```python
from build123d import *

# Parameters (mm, degrees)
SKETCH_2_R          = 40
EXTRUDE_1_DEPTH     = 40
SKETCH_1_R          = 16.5
CUT_EXTRUDE_1_DEPTH = 30
EXTRUDE_2_DEPTH     = 15
SKETCH_4_W          = 12
SKETCH_4_H          = 7.528633981
CUT_EXTRUDE_2_DEPTH = 30


with BuildPart() as part:
    # 草图2 → 凸台-拉伸1 (new body)
    with BuildSketch(Plane.XY):
        Circle(SKETCH_2_R)
    extrude(amount=EXTRUDE_1_DEPTH)

    # 草图1 → 切除-拉伸1 (cut)
    with BuildSketch(Plane.XY):
        Circle(SKETCH_1_R)
    extrude(amount=CUT_EXTRUDE_1_DEPTH, mode=Mode.SUBTRACT)

    # 草图3 → 凸台-拉伸2 (add)
    with BuildSketch(Plane.XY.offset(40)):
        with BuildLine():
            Line((22.230762114, 21.495190528), (29.730762114, 8.504809472))
            Line((29.730762114, 8.504809472), (37.776643972, 13.150101528))
            ThreePointArc((37.776643972, 13.150101528), (34.641016151, 20), (30.276643972, 26.140482585))
            Line((30.276643972, 26.140482585), (22.230762114, 21.495190528))
        make_face()
        with BuildLine():
            Line((-7.5, 39.290584114), (-7.5, 30))
            Line((-7.5, 30), (7.5, 30))
            Line((7.5, 30), (7.5, 39.290584114))
            ThreePointArc((7.5, 39.290584114), (0, 40), (-7.5, 39.290584114))
        make_face()
        with BuildLine():
            Line((29.730762114, -8.504809472), (22.230762114, -21.495190528))
            Line((22.230762114, -21.495190528), (30.276643972, -26.140482585))
            ThreePointArc((30.276643972, -26.140482585), (34.641016151, -20), (37.776643972, -13.150101528))
            Line((37.776643972, -13.150101528), (29.730762114, -8.504809472))
        make_face()
        with BuildLine():
            Line((7.5, -30), (-7.5, -30))
            Line((-7.5, -30), (-7.5, -39.290584114))
            ThreePointArc((-7.5, -39.290584114), (0, -40), (7.5, -39.290584114))
            Line((7.5, -39.290584114), (7.5, -30))
        make_face()
        with BuildLine():
            Line((-22.230762114, -21.495190528), (-29.730762114, -8.504809472))
            Line((-29.730762114, -8.504809472), (-37.776643972, -13.150101528))
            ThreePointArc((-37.776643972, -13.150101528), (-34.641016151, -20), (-30.276643972, -26.140482585))
            Line((-30.276643972, -26.140482585), (-22.230762114, -21.495190528))
        make_face()
        with BuildLine():
            Line((-29.730762114, 8.504809472), (-22.230762114, 21.495190528))
            Line((-22.230762114, 21.495190528), (-30.276643972, 26.140482585))
            ThreePointArc((-30.276643972, 26.140482585), (-34.641016151, 20), (-37.776643972, 13.150101528))
            Line((-37.776643972, 13.150101528), (-29.730762114, 8.504809472))
        make_face()
    extrude(amount=EXTRUDE_2_DEPTH)

    # 草图4 → 切除-拉伸2 (cut)
    with BuildSketch(Plane(origin=(0, 0, 0), x_dir=(-1, 0, 0), z_dir=(0, 0, -1))):
        with Locations((0, 15.23568301)):
            Rectangle(SKETCH_4_W, SKETCH_4_H)
    extrude(amount=-CUT_EXTRUDE_2_DEPTH, mode=Mode.SUBTRACT)


solid = part.part
```
Geometry check sheet. Reference: the model listing, model coordinates, mm. A direction names the side the tool comes from. Round coordinates to 2 decimals unless told otherwise and drop trailing zeros. Order: outer loops, then holes, each group sorted by start corner. A loop starts at its lowest first (then second) coordinate and runs counter-clockwise, first axis right, second up. Notation, with made-up numbers: (21, 86.5) - (57, 86.5) arc R34 cw to (57, 116.5) - close; hole circle Ø2 at (-39, 86.25). An arc over 180 degrees is marked (long way). Use a Markdown table: item, result. Add a question column.
(1) Release check for a two-part mould opening along Y. For faces 1 (the flat face through (7.5, -35, 47)), 2 (the flat face through (0, 1, 30)), 3 (the flat face through (-26.197, 23.785, 47.395)), 4 (the flat face through (-26.033, 14.909, 47.395)) record: pulls with the +Y half, pulls with the -Y half, needs draft (parallel to the pull), parting line crosses it, or undercut.
(2) Depth check by flat-ended pin: pin 1 (6 mm diameter, centred on y = 1, z = 40, fed in from -X); pin 2 (12 mm diameter, centred on x = -2.5, y = 0.5, fed in from -Z); pin 3 (6 mm diameter, centred on x = -1.5, z = 12.5, fed in from -Y). Enter the tip coordinate at first touch or a pass-through.
(3) Tool access check on faces 5 (the flat face through (7.5, 35, 47)), 6 (the flat face through (-7.5, -35, 47)), 7 (the flat face through (26.033, -14.909, 47.395)), 8 (the flat face through (-33.697, -10.795, 47.395)). Record the directions out of +Z, -Z, +X, -X, +Y, -Y that give a thin tool (end or side, any length) a straight path to the whole face; none if there is none.
(4) Sectioned sample at B-B, the plane x = 0. Enter the section's corners in (y, z).
(5) Sectioned sample at D-D, the plane y = -24.5. Enter the section's corners in (x, z).
(6) Sectioned sample at A-A, the plane y = 0. Enter the section's corners in (x, z), and give its area (3 significant figures).
(7) Sectioned sample at C-C, the plane x = 27. Enter the section's corners in (y, z).
(8) Material ranges on line 1 along X through (y, z) = (0, 21); line 2 along Y through (x, z) = (0, 9); line 3 along Z through (x, y) = (-26, 9.5), recorded low to high. Write a range as [from, to].
Answers below:
| question | item | result |
|---|---|---|
| 1 | face 1 | needs draft |
| 1 | face 2 | undercut |
| 1 | face 3 | pulls with the +Y half |
| 1 | face 4 | undercut |
| 2 | pin 1 | x = -40 |
| 2 | pin 2 | z = 30 |
| 2 | pin 3 | y = -40 |
| 3 | face 5 | +Z, +X, +Y, -Y |
| 3 | face 6 | +Z, -X, +Y, -Y |
| 3 | face 7 | +Z |
| 3 | face 8 | +Z, -X |
| 4 | outline | (-40, 0) - (-16.5, 0) - (-16.5, 30) - (19, 30) - (19, 0) - (40, 0) - (40, 55) - (30, 55) - (30, 40) - (-30, 40) - (-30, 55) - (-40, 55) - close |
| 5 | outline | (-31.62, 0) - (31.62, 0) - (31.62, 55) - (27.44, 55) - (27.44, 40) - (-27.44, 40) - (-27.44, 55) - (-31.62, 55) - close |
| 6 | outline | (-40, 0) - (-16.5, 0) - (-16.5, 30) - (16.5, 30) - (16.5, 0) - (40, 0) - (40, 40) - (-40, 40) - close |
| 6 | area | 2,210 mm² |
| 7 | outline | (-29.51, 0) - (29.51, 0) - (29.51, 40) - (24.25, 40) - (24.25, 55) - (13.23, 55) - (13.23, 40) - (-13.23, 40) - (-13.23, 55) - (-24.25, 55) - (-24.25, 40) - (-29.51, 40) - close |
| 8 | line 1 | [-40, -16.5], [16.5, 40] |
| 8 | line 2 | [-40, -16.5], [19, 40] |
| 8 | line 3 | [0, 40] |
